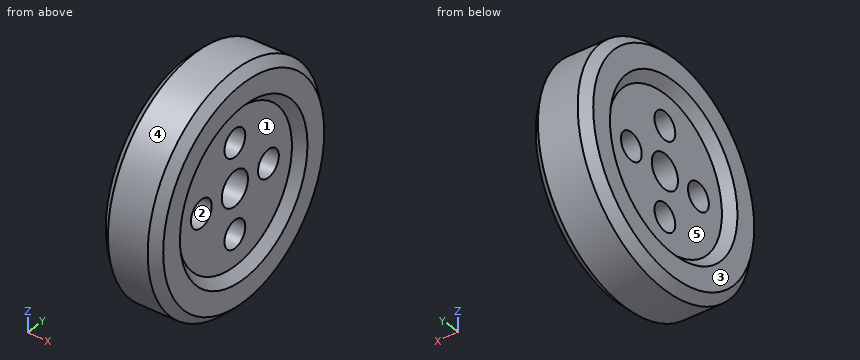
from build123d import *

# Parameters (mm, degrees)
THREAD_HOLES_5X_REACH = 385.797
THREAD_HOLES_SKETCH_R = 31


with BuildPart() as part:
    # Disc Profile Sketch → Button Disc Body (revolve)
    with BuildSketch(Plane.XY, mode=Mode.PRIVATE) as button_disc_body_sk:
        Polygon((-45, 260), (-65, 240), (-65, 190), (-45, 170), (-45, 39), (45, 39), (45, 170), (65, 190), (65, 240), (45, 260), align=None)
    revolve(button_disc_body_sk.sketch.rotate(Axis((-186.115918114, 0, 0), (1, 0, 0)), 90), axis=Axis((-186.115918114, 0, 0), (1, 0, 0)))

    # Thread Holes Sketch → Thread Holes 5x (cut, up to next)
    with BuildSketch(Plane(origin=(45, 0, 0), x_dir=(0, 0, -1), z_dir=(1, 0, 0)), mode=Mode.PRIVATE) as thread_holes_5x_sk1:
        with Locations((0, 100)):
            Circle(THREAD_HOLES_SKETCH_R)
    thread_holes_5x_tool1 = extrude(thread_holes_5x_sk1.sketch, amount=-THREAD_HOLES_5X_REACH, mode=Mode.PRIVATE) & part.part
    # Thread Holes Sketch → Thread Holes 5x (cut, up to next)
    with BuildSketch(Plane(origin=(45, 0, 0), x_dir=(0, 0, -1), z_dir=(1, 0, 0)), mode=Mode.PRIVATE) as thread_holes_5x_sk2:
        with Locations((100, 0)):
            Circle(THREAD_HOLES_SKETCH_R)
    thread_holes_5x_tool2 = extrude(thread_holes_5x_sk2.sketch, amount=-THREAD_HOLES_5X_REACH, mode=Mode.PRIVATE) & part.part
    # Thread Holes Sketch → Thread Holes 5x (cut, up to next)
    with BuildSketch(Plane(origin=(45, 0, 0), x_dir=(0, 0, -1), z_dir=(1, 0, 0)), mode=Mode.PRIVATE) as thread_holes_5x_sk3:
        with Locations((0, -100)):
            Circle(THREAD_HOLES_SKETCH_R)
    thread_holes_5x_tool3 = extrude(thread_holes_5x_sk3.sketch, amount=-THREAD_HOLES_5X_REACH, mode=Mode.PRIVATE) & part.part
    # Thread Holes Sketch → Thread Holes 5x (cut, up to next)
    with BuildSketch(Plane(origin=(45, 0, 0), x_dir=(0, 0, -1), z_dir=(1, 0, 0)), mode=Mode.PRIVATE) as thread_holes_5x_sk4:
        with Locations((-100, 0)):
            Circle(THREAD_HOLES_SKETCH_R)
    thread_holes_5x_tool4 = extrude(thread_holes_5x_sk4.sketch, amount=-THREAD_HOLES_5X_REACH, mode=Mode.PRIVATE) & part.part
    add(thread_holes_5x_tool1.solids().sort_by_distance((45, 100, 0))[0], mode=Mode.SUBTRACT)
    add(thread_holes_5x_tool2.solids().sort_by_distance((45, 0, -100))[0], mode=Mode.SUBTRACT)
    add(thread_holes_5x_tool3.solids().sort_by_distance((45, -100, 0))[0], mode=Mode.SUBTRACT)
    add(thread_holes_5x_tool4.solids().sort_by_distance((45, 0, 100))[0], mode=Mode.SUBTRACT)


solid = part.part
The model under review builds one solid part; all positions refer to its coordinate system, in mm. Face numbers are marked on the shaded views. A direction names the side the tool comes from. Coordinates: 2 decimals unless noted, no trailing zeros. Loops run counter-clockwise (first coordinate to the right, second up) from the corner with the lowest first, then second, coordinate; pieces in that order, holes last. Notation, with made-up numbers: (14.25, 68.25) -> (48.25, 68.25) arc R34 ccw to (48.25, 101.25) -> close; hole circle Ø3 at (15, -39.5). An arc over 180 degrees is marked (long way). Use a Markdown table: item, result. Add a question column.
1. Clearance check with flat-ended pins moving along their axes: pin 1 Ø2 at (x, z) = (-38, -64) entering from -Y; pin 2 Ø1 at (y, z) = (-46, 6) entering from -X; pin 3 Ø6 at (x, z) = (39, 34) entering from +Y. State where each tip first meets the part, or that it passes through.
2. To check wall thickness, follow line 1 (Y direction, x = 4, z = 0); line 2 (Y direction, x = -21, z = 100); line 3 (Z direction, x = 32.5, y = 10). State the ranges of each line that lie inside material, in increasing order.
3. Machinability: for the marked faces 1 and 2, which of the approach directions +Z, -Z, +X, -X, +Y, -Y give a long, thin tool a straight path to every point of the face, cutting with its end or side? Answer none if there is none.
4. Draft analysis for pull direction Z (two halves, no side actions). For the marked faces 3, 4 and 5, state which applies: pulls with the +Z half, pulls with the -Z half, needs draft (parallel to the pull), parting line crosses it, or undercut.
5. Add section C-C on x = 13.5. Write out the cut boundary in (y, z).
6. Add section A-A on y = 0. Write out the cut boundary in (x, z).
Returned:
| question | item | result |
|---|---|---|
| 1 | pin 1 | stops at y = -252.25 |
| 1 | pin 2 | stops at x = -45 |
| 1 | pin 3 | stops at y = 258.15 |
| 2 | line 1 | y = -260 to -131, -69 to -39, 39 to 69, 131 to 260 |
| 2 | line 2 | y = -240 to -31, 31 to 240 |
| 2 | line 3 | z = -259.81 to -129.34, -70.66 to -37.7, 37.7 to 70.66, 129.34 to 259.81 |
| 3 | face 1 | +X |
| 3 | face 2 | +X, -X |
| 4 | face 3 | needs draft |
| 4 | face 4 | parting line crosses it |
| 4 | face 5 | undercut |
| 5 | outline | circle Ø520 at (0, 0); hole circle Ø62 at (-100, 0); hole circle Ø78 at (0, 0); hole circle Ø62 at (0, -100); hole circle Ø62 at (0, 100); hole circle Ø62 at (100, 0) |
| 6 | outline | (-65, -240) -> (-45, -260) -> (45, -260) -> (65, -240) -> (65, -190) -> (45, -170) -> (45, -131) -> (-45, -131) -> (-45, -170) -> (-65, -190) -> close; (-65, 190) -> (-45, 170) -> (-45, 131) -> (45, 131) -> (45, 170) -> (65, 190) -> (65, 240) -> (45, 260) -> (-45, 260) -> (-65, 240) -> close; (-45, -69) -> (45, -69) -> (45, -39) -> (-45, -39) -> close; (-45, 39) -> (45, 39) -> (45, 69) -> (-45, 69) -> close |
